from build123d import *

# Parameters (mm, degrees)
BOSS_EXTRUDE1_DEPTH = 8
SKETCH2_R           = 7
BOSS_EXTRUDE2_DEPTH = 114
CHAMFER1_SIZE       = 2
SCALE_1_SCALE       = 1.875


with BuildPart() as part:
    # Sketch1 → Boss-Extrude1 (new body)
    with BuildSketch(Plane(origin=(0, 0, 0), x_dir=(1, 0, 0), z_dir=(0, 1, 0))):
        Polygon((12.124355653, 0), (6.062177826, 10.5), (-6.062177826, 10.5), (-12.124355653, 0), (-6.062177826, -10.5), (6.062177826, -10.5), align=None)
    extrude(amount=BOSS_EXTRUDE1_DEPTH)

    # Sketch2 → Boss-Extrude2 (add)
    with BuildSketch(Plane(origin=(0, 8, 0), x_dir=(1, 0, 0), z_dir=(0, 1, 0))):
        with Locations(Location((0, 0, 0), (0, 0, 90))):
            Circle(SKETCH2_R)
    extrude(amount=BOSS_EXTRUDE2_DEPTH)

    # Chamfer1
    chamfer1_edges = [part.edges().sort_by_distance(p)[0] for p in [
        (0, 122, 7),
    ]]
    chamfer(chamfer1_edges, length=CHAMFER1_SIZE)

    # Sketch3 → Cut-Revolve1 (revolve, cut)
    with BuildSketch(Plane.XY, mode=Mode.PRIVATE) as cut_revolve1_sk:
        with BuildLine():
            Line((-12.124355653, 0), (-12.124355653, 1))
            ThreePointArc((-12.124355653, 1), (-10.705494483, 0.25658351), (-9.124355653, 0))
            Line((-9.124355653, 0), (-12.124355653, 0))
        make_face()
    revolve(cut_revolve1_sk.sketch.rotate(Axis((0, 0, 0), (0, 1, 0)), 270), axis=Axis((0, 0, 0), (0, 1, 0)), mode=Mode.SUBTRACT)


with BuildPart() as part_1:
    # Scale 1: scaled about (-1.43e-07, 55.752743575, -2.4e-08)
    add(part.part.scale(SCALE_1_SCALE).moved(Location((1.25e-07, -48.783650628, 2.1e-08))))


solid = part_1.part
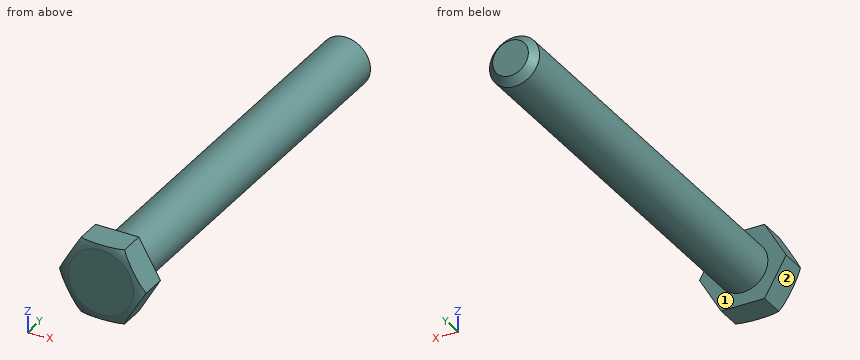
Read the model definition and answer for the solid it produces. Units are mm, in the model's axes. Face numbers are marked on the shaded views. A direction names the side the tool comes from. Coordinates: 2 decimals unless noted, no trailing zeros. Write each loop counter-clockwise with the first axis right and the second up, starting at its lowest first coordinate (ties: lowest second). Pieces come first, ordered by that corner, then holes. Notation, with made-up numbers: M 33,58 L 81,58 A16 cw 81,69 Z; hole C 19,66.25 d1. An arc over 180 degrees is marked long. Use a Markdown table: item, result.
Q1. Each of these flat-tipped pins is pushed along its axis until it touches: pin 1 Ø1 at (y, z) = (16.5, -15.5) entering from +X; pin 2 Ø12 at (y, z) = (-21, -12.5) entering from +X; pin 3 Ø3 at (y, z) = (99, -9) entering from +X; pin 4 Ø1.5 at (x, y) = (-6, -24.5) entering from +Z. Where does it stop, or does it pass through?
Answer block:
| item | result |
|---|---|
| pin 1 | passes through |
| pin 2 | stops at x = 11.4 |
| pin 3 | stops at x = 10.77 |
| pin 4 | stops at z = 12.03 |
Q2. Straight lines are drawn through the part: L1, parallel to Y at x = -15.5, z = 7; L2, parallel to Z at x = 0.5, y = 37; L3, parallel to X at y = 52.5, z = -1.5. For each, find the intervals that lie inside material, in ascending order. Write a range as [from, to].
Answer block:
| item | result |
|---|---|
| L1 | y = [-48.78, -33.78] |
| L2 | z = [-13.12, 13.12] |
| L3 | x = [-13.04, 13.04] |
Q3. The part is cut by section A-A, the plane y = 46. Write down the section's boundary in (x, z) (3 decimals), then the cut area to 3 significant figures.
Answer block:
| item | result |
|---|---|
| outline | C 0,0 d26.25 |
| area | 541 mm2 |
Q4. Which of the six approach directions +Z, -Z, +X, -X, +Y, -Y give full straight-line access (tool end or side, diameter ignored) to the marked faces 1 and 2?
Answer block:
| item | result |
|---|---|
| face 1 | +Y |
| face 2 | -Z, -X, +Y, -Y |
